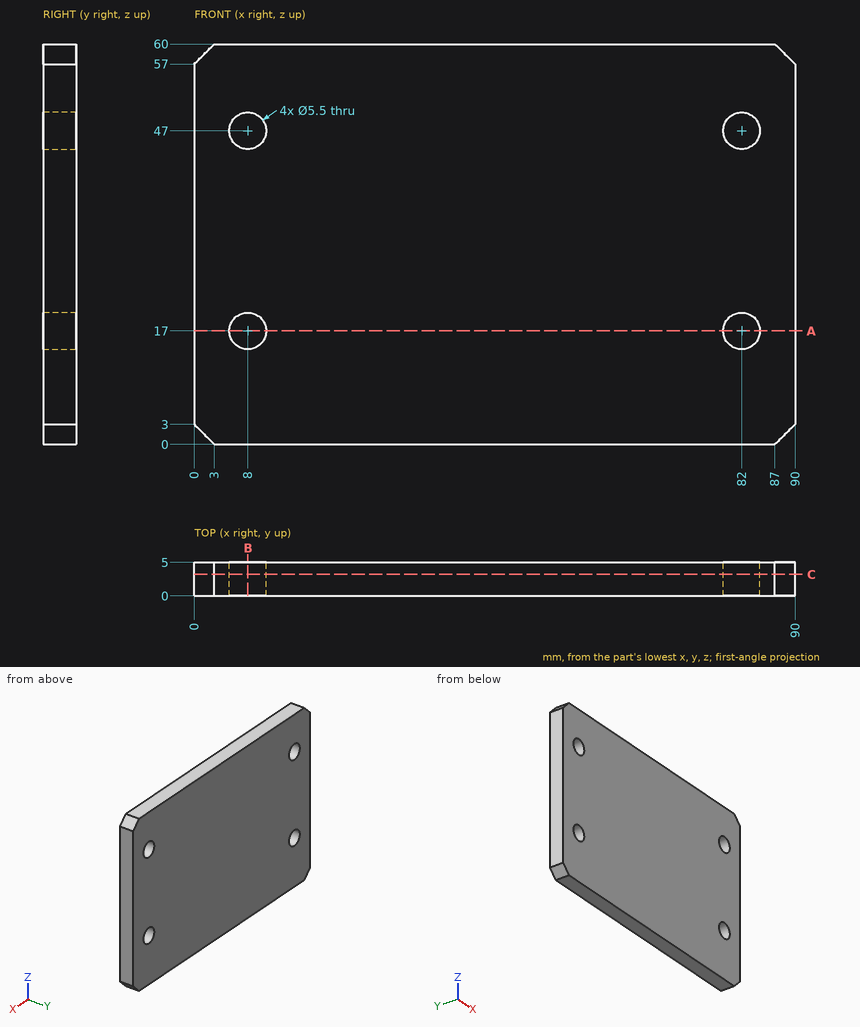
Design review of the part shown in the three views and the two pictorial views. Dimensions are in mm from the part's minimum x, y and z. Give positions to 0.01 mm unless a question says otherwise; leave off trailing zeros. Loops run counter-clockwise (first coordinate to the right, second up) from the corner with the lowest first, then second, coordinate; pieces in that order, holes last. Notation, with made-up numbers: (-2.75, 27.25) -> (47.25, 27.25) arc R21 cw to (47.25, 51.25) -> close; hole circle Ø7 at (57.5, 27.5). An arc over 180 degrees is marked (long way). Answer as a JSON object with one key per item and string values. Group by question number.
Q1. Wall thickness on line 1 along X through (y, z) = (1.55, 17); line 2 along Z through (x, y) = (82, 2.5); line 3 along X through (y, z) = (0.9, 15): over which ranges is each line inside the solid? List them lowest first.
Q2. Take a section at B-B (x = 8). Write out the cut boundary in (y, z).
Q3. Insertion check: pin 1 (9 mm diameter, centred on x = 82, z = 47, fed in from -Y); pin 2 (5 mm diameter, centred on x = 8, z = 47, fed in from +Y). Each pin has a flat end and moves straight along its axis. Give the tip position at first contact, or say it passes through.
Q4. Take a section at C-C (y = 3.2). Write out the cut boundary in (x, z), plus the area to 3 significant figures.
Q5. Take a section at A-A (z = 17). Write out the cut boundary in (x, y).
Answer below:
{
 "1": {"line 1": "x = 0 to 5.25, 10.75 to 79.25, 84.75 to 90", "line 2": "z = 0 to 14.25, 19.75 to 44.25, 49.75 to 60", "line 3": "x = 0 to 6.11, 9.89 to 80.11, 83.89 to 90"},
 "2": {"outline": "(0, 0) -> (5, 0) -> (5, 14.25) -> (0, 14.25) -> close; (0, 19.75) -> (5, 19.75) -> (5, 44.25) -> (0, 44.25) -> close; (0, 49.75) -> (5, 49.75) -> (5, 60) -> (0, 60) -> close"},
 "3": {"pin 1": "stops at y = 0", "pin 2": "passes through"},
 "4": {"outline": "(0, 3) -> (3, 0) -> (87, 0) -> (90, 3) -> (90, 57) -> (87, 60) -> (3, 60) -> (0, 57) -> close; hole circle Ø5.5 at (8, 17); hole circle Ø5.5 at (8, 47); hole circle Ø5.5 at (82, 17); hole circle Ø5.5 at (82, 47)", "area": "5,290 mm2"},
 "5": {"outline": "(0, 0) -> (5.25, 0) -> (5.25, 5) -> (0, 5) -> close; (10.75, 0) -> (79.25, 0) -> (79.25, 5) -> (10.75, 5) -> close; (84.75, 0) -> (90, 0) -> (90, 5) -> (84.75, 5) -> close"}
}
